from build123d import *

# Parameters (mm, degrees)
SKETCH_1_W              = 12.5
SKETCH_1_H              = 90
EXTRUDE_1_DEPTH         = 90
CHAMFER_1_SIZE          = 3
HOLE_WIZARD_M8_1_D      = 6.8
SKETCH_6_R              = 14
CUT_EXTRUDE_1_DEPTH     = 8
SKETCH_7_R              = 12
CUT_EXTRUDE_2_DEPTH     = 128.530388535
CHAMFER_2_SIZE          = 0.5
SKETCH_10_W             = 12.5
SKETCH_10_H             = 15
EXTRUDE_3_DEPTH         = 15
SKETCH_11_W             = 12.5
SKETCH_11_H             = 15
EXTRUDE_4_DEPTH         = 15
CHAMFER_4_SIZE          = 2
HOLE_WIZARD_6_5_6_5_1_D = 6.5


with BuildPart() as part:
    # 草图1 → 凸台-拉伸1 (new body)
    with BuildSketch(Plane(origin=(0, 0, 0), x_dir=(0, 0, -1), z_dir=(1, 0, 0))):
        with Locations((6.25, 45)):
            Rectangle(SKETCH_1_W, SKETCH_1_H)
    extrude(amount=EXTRUDE_1_DEPTH)

    # 倒角1
    chamfer_1_edges = [part.edges().sort_by_distance(p)[0] for p in [
        (90, 90, -6.25),
        (0, 90, -6.25),
    ]]
    chamfer(chamfer_1_edges, length=CHAMFER_1_SIZE)

    # M8 螺纹孔1 (through all)
    with Locations(Plane(origin=(0, 0, -12.5), x_dir=(-1, 0, 0), z_dir=(0, 0, -1))):
        with Locations((-15, 75), (-75, 75)):
            Hole(HOLE_WIZARD_M8_1_D / 2)

    # 草图6 → 切除-拉伸1 (cut)
    with BuildSketch(Plane.XY):
        with Locations((45, 40)):
            Circle(SKETCH_6_R)
    extrude(amount=-CUT_EXTRUDE_1_DEPTH, mode=Mode.SUBTRACT)

    # 草图7 → 切除-拉伸2 (cut, through all)
    with BuildSketch(Plane.XY.offset(-8)):
        with Locations((45, 40)):
            Circle(SKETCH_7_R)
    extrude(amount=-CUT_EXTRUDE_2_DEPTH, mode=Mode.SUBTRACT)

    # 倒角2
    chamfer_2_edges = [part.edges().sort_by_distance(p)[0] for p in [
        (31, 40, 0),
        (33, 40, -12.5),
    ]]
    chamfer(chamfer_2_edges, length=CHAMFER_2_SIZE)

    # 草图10 → 凸台-拉伸3 (add)
    with BuildSketch(Plane(origin=(90, 0, 0), x_dir=(0, 0, -1), z_dir=(1, 0, 0))):
        with Locations((6.25, 7.5)):
            Rectangle(SKETCH_10_W, SKETCH_10_H)
    extrude(amount=EXTRUDE_3_DEPTH)

    # 草图11 → 凸台-拉伸4 (add)
    with BuildSketch(Plane.ZY):
        with Locations((-6.25, 7.5)):
            Rectangle(SKETCH_11_W, SKETCH_11_H)
    extrude(amount=EXTRUDE_4_DEPTH)

    # 倒角4
    chamfer_4_edges = [part.edges().sort_by_distance(p)[0] for p in [
        (105, 7.5, 0),
        (-15, 7.5, 0),
        (-15, 7.5, -12.5),
        (105, 7.5, -12.5),
    ]]
    chamfer(chamfer_4_edges, length=CHAMFER_4_SIZE)

    # Ø6.5 (6.5) 直径孔1 (through all)
    with Locations(Plane(origin=(-61.758148559, 15, 1.949959902), x_dir=(1, 0, 0), z_dir=(0, 1, 0))):
        with Locations((159.258148559, 8.199959902), (54.258148559, 8.199959902)):
            Hole(HOLE_WIZARD_6_5_6_5_1_D / 2)


solid = part.part
The listing builds one solid part. Answer for the finished solid, in the listing's coordinates (mm). A direction names the side the tool comes from. Round coordinates to 2 decimals unless told otherwise and drop trailing zeros. Write each loop counter-clockwise with the first axis right and the second up, starting at its lowest first coordinate (ties: lowest second). Pieces come first, ordered by that corner, then holes. Notation, with made-up numbers: (2.5, -8) - (56.5, -8) arc R8 ccw to (56.5, 4) - close; hole circle Ø5 at (-22.75, 20.5). An arc over 180 degrees is marked (long way). Use a Markdown table: item, result. Add a question column.
1. For a pull along X with two mould halves and no side action, classify faces 1 (the face through (41.97, 26.33, -4.2)), 2 (the face through (1, 88, -6)), 3 (the face through (96, 15, -3)) as +X half, -X half, draft (parallel to the pull), parting line (faces both ways), or undercut.
2. The part is cut by section D-D (y = 85.5). Write down the section's boundary in (x, z).
3. The part is cut by section C-C (x = 97.5). Write down the section's boundary in (y, z), and give its area (3 significant figures).
4. Consider line 1 (Y direction, x = 15, z = -6.75); line 2 (Z direction, x = -7.5, y = 4); line 3 (Y direction, x = 45, z = -6). Determine where each line is inside the solid, lowest interval first.
5. The part is cut by section B-B (y = 40). Write down the section's boundary in (x, z), and give its area (4 significant figures).
6. The part is cut by section A-A (x = 75). Write down the section's boundary in (y, z), and give its area (3 significant figures).
7. Flat-ended cylindrical pins translate along their axes: P1, Ø4, axis at y = 47, z = -4, coming from the +X side; P2, Ø4, axis at x = -7.5, z = -4, coming from the +Y side; P3, Ø6, axis at y = 31.5, z = -4.5, coming from the -X side. Find the tip coordinate at first contact, or state that the pin passes through.
8. A tool of negligible diameter and unlimited length cuts with its end or side. For faces 4 (the face through (100.747, 7.395, -6.393)), 5 (the face through (90, 52, -6)), 6 (the face through (38.7, 50.4, -8)), 7 (the face through (0, 52, -6)), 8 (the face through (59, 34, 0)), from which of +Z, -Z, +X, -X, +Y, -Y can it reach the whole face along a straight path? Write none if from no direction.
Reported:
| question | item | result |
|---|---|---|
| 1 | face 1 | undercut |
| 1 | face 2 | -X half |
| 1 | face 3 | draft |
| 2 | outline | (0, -12.5) - (90, -12.5) - (90, 0) - (0, 0) - close |
| 3 | outline | (0, -12.5) - (15, -12.5) - (15, -9.5) - (0, -9.5) - close; (0, -3) - (15, -3) - (15, 0) - (0, 0) - close |
| 3 | area | 90.0 mm^2 |
| 4 | line 1 | 0 to 71.6, 78.4 to 90 |
| 4 | line 2 | -12.5 to -9.5, -3 to 0 |
| 4 | line 3 | 0 to 26, 54 to 90 |
| 5 | outline | (0, -12.5) - (32.5, -12.5) - (33, -12) - (33, -8) - (31, -8) - (31, -0.5) - (30.5, 0) - (0, 0) - close; (57, -12) - (57.5, -12.5) - (90, -12.5) - (90, 0) - (59.5, 0) - (59, -0.5) - (59, -8) - (57, -8) - close |
| 5 | area | 792.5 mm^2 |
| 6 | outline | (0, -12.5) - (71.6, -12.5) - (71.6, 0) - (0, 0) - close; (78.4, -12.5) - (90, -12.5) - (90, 0) - (78.4, 0) - close |
| 6 | area | 1,040 mm^2 |
| 7 | P1 | x = 90 |
| 7 | P2 | y = 15 |
| 7 | P3 | x = 0 |
| 8 | face 4 | +Y, -Y |
| 8 | face 5 | +Z, -Z, +X, +Y |
| 8 | face 6 | +Z |
| 8 | face 7 | +Z, -Z, -X, +Y |
| 8 | face 8 | +Z, +X, -X, +Y, -Y |
